The drawing under review shows one solid part. Ordinate dimensions are in mm from its lowest x, y, z. A direction names the side the tool comes from. Coordinates: 2 decimals unless noted, no trailing zeros. Order: outer loops, then holes, each group sorted by start corner. A loop starts at its lowest first (then second) coordinate and runs counter-clockwise, first axis right, second up. Notation, with made-up numbers: (9, 0) - (34, 0) arc R20 cw to (34, 7) - close; hole circle Ø6 at (59.25, 35.25). An arc over 180 degrees is marked (long way). Write each question's results on one line, items separated by ' | '. Start each with the question number.
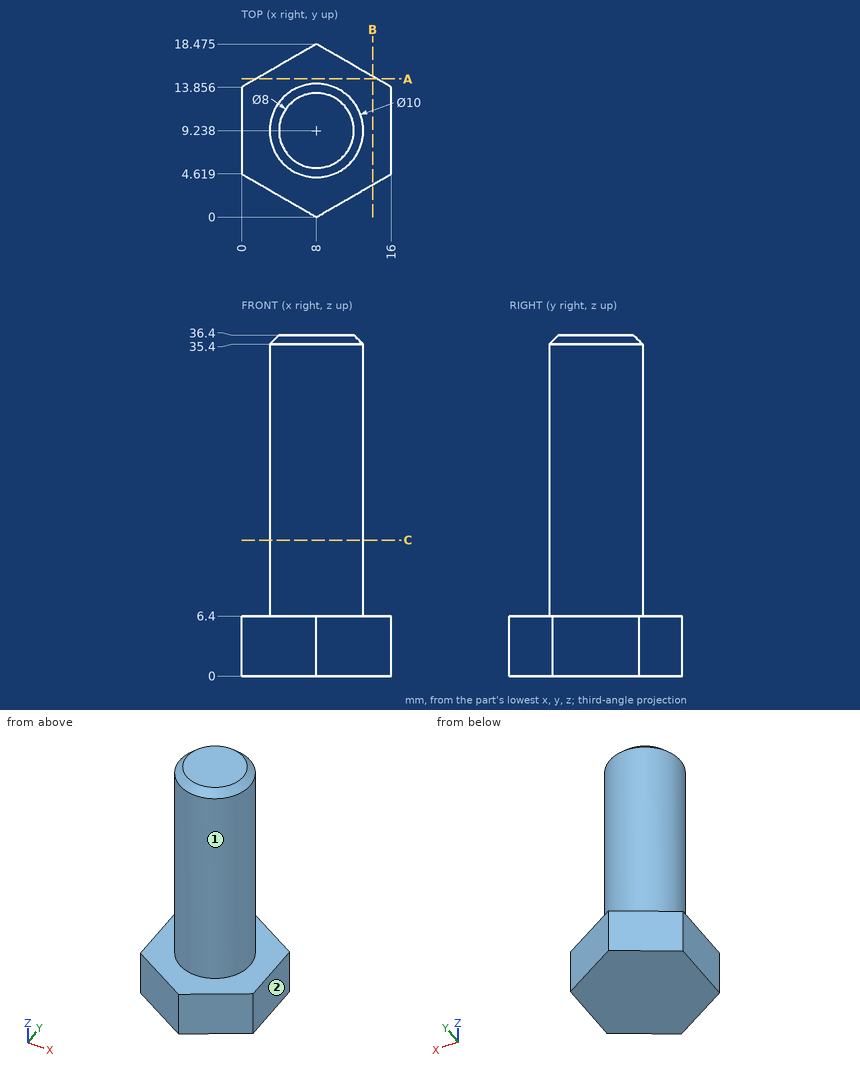
(1) Take a section at C-C (z = 14.5). State the section outline as (x, y) points.
(2) Take a section at A-A (y = 14.75). State the section outline as (x, z) points.
(3) To check wall thickness, follow line 1 along Z through (x, y) = (14.5, 8.75); line 2 along Y through (x, z) = (8, 7); line 3 along Y through (x, z) = (11, 28). State the ranges of each line that lie inside material, in increasing order. Write a range as [from, to].
(4) Take a section at B-B (x = 14). State the section outline as (y, z) points.
(5) Clearance check with flat-ended pins moving along their axes: pin 1 (3 mm diameter, centred on x = 3, z = 6.5, fed in from -Y); pin 2 (3 mm diameter, centred on y = 4, z = 29.5, fed in from +X); pin 3 (1 mm diameter, centred on y = 3.5, z = 24.5, fed in from +X); pin 4 (1.5 mm diameter, centred on y = 12.5, z = 21.5, fed in from -X). State where each tip first meets the part, or that it passes through.
(6) Tool access review of the marked faces 1 and 2: name each direction out of +Z, -Z, +X, -X, +Y, -Y from which nothing blocks a thin tool from reaching the whole face with its end or side.
Worked out:
1) outline: circle Ø10 at (8, 9.24)
2) outline: (1.55, 0) - (14.45, 0) - (14.45, 6.4) - (1.55, 6.4) - close
3) line 1: [0, 6.4] | line 2: [4.24, 14.24] | line 3: [5.24, 13.24]
4) outline: (3.46, 0) - (15.01, 0) - (15.01, 6.4) - (3.46, 6.4) - close
5) pin 1: y = 2.02 | pin 2: x = 11.32 | pin 3: through | pin 4: x = 3.68
6) face 1: +Z | face 2: +Z, -Z, +X, +Y, -Y
